Design review of the part built by this model. Coordinates are the model's own, in mm. A direction names the side the tool comes from. Round coordinates to 2 decimals unless told otherwise and drop trailing zeros. Order: outer loops, then holes, each group sorted by start corner. A loop starts at its lowest first (then second) coordinate and runs counter-clockwise, first axis right, second up. Notation, with made-up numbers: M 61,42.5 L 114,42.5 A14 ccw 114,51.5 Z; hole C -21.75,34 d8. An arc over 180 degrees is marked long. Write each question's results on one line, items separated by ' | '. Start each with the question number.
Item 1: Clearance check with flat-ended pins moving along their axes: pin 1 (1.5 mm diameter, centred on x = -3.5, y = 114, fed in from -Z); pin 2 (10 mm diameter, centred on x = 7, y = 132, fed in from +Z); pin 3 (5 mm diameter, centred on x = -8.5, y = 6.5, fed in from +Z); pin 4 (9 mm diameter, centred on x = -0.5, z = -3, fed in from -Y). State where each tip first meets the part, or that it passes through.
Item 2: Machinability: for faces 1 (the flat face through (10, -10, 0)), 2 (the flat face through (1, 0, -11)), 3 (the cylindrical face through (-1.951, -28.786, 19.86)), 4 (the flat face through (0, -8, -10)), 5 (the cylindrical face through (0.66, 93.67, -14.985)), which of the approach directions +Z, -Z, +X, -X, +Y, -Y give a long, thin tool a straight path to every point of the face, cutting with its end or side? Answer none if there is none.
Item 3: Wall thickness on line 1 (X direction, y = -5.5, z = -6); line 2 (Y direction, x = 2, z = -11.5); line 3 (Z direction, x = 0.5, y = 38): over which ranges is each line inside the solid? List them lowest first. Write a range as [from, to].
Item 4: Take a section at B-B, the plane x = 0. Write out the cut boundary in (y, z), plus the area to 3 significant figures.
Item 5: Take a section at C-C, the plane y = 39. Write out the cut boundary in (x, z).
Item 6: Take a section at D-D, the plane z = -19. Write out the cut boundary in (x, y).
Item 7: Take a section at A-A, the plane z = 0. Write out the cut boundary in (x, y), plus the area to 3 significant figures.
```python
from build123d import *

# Parameters (mm, degrees)
SKETCH_1_R           = 15
EXTRUDE_1_DEPTH      = 190
EXTRUDE_2_DEPTH      = 10
EXTRUDE_2_DEPTH_BACK = 10
EXTRUDE_3_DEPTH      = 20
EXTRUDE_3_DEPTH_BACK = 40
SKETCH_3_R           = 9


with BuildPart() as part:
    # 草图1 → 凸台-拉伸1 (new body)
    with BuildSketch(Plane(origin=(0, 0, 0), x_dir=(1, 0, 0), z_dir=(0, 1, 0))):
        with Locations(Location((0, 0, 0), (0, 0, 270))):
            Circle(SKETCH_1_R)
    extrude(amount=EXTRUDE_1_DEPTH)

    # 草图2 → 凸台-拉伸2 (add, two sides: drawn at the far end of the back side and taken through both)
    with BuildSketch(Plane.XY.offset(-EXTRUDE_2_DEPTH_BACK)):
        with BuildLine():
            Line((10, 0), (10, -20))
            ThreePointArc((10, -20), (0, -30), (-10, -20))
            Line((-10, -20), (-10, 0))
            ThreePointArc((-10, 0), (0, 10), (10, 0))
        make_face()
    extrude(amount=EXTRUDE_2_DEPTH + EXTRUDE_2_DEPTH_BACK)

    # 草图3 → 凸台-拉伸3 (add, two sides: drawn at the far end of the back side and taken through both)
    with BuildSketch(Plane.XY.offset(10).offset(-EXTRUDE_3_DEPTH_BACK)):
        with Locations((0, -20)):
            Circle(SKETCH_3_R)
    extrude(amount=EXTRUDE_3_DEPTH + EXTRUDE_3_DEPTH_BACK)


solid = part.part
```
Results list:
1) pin 1: z = -14.75 | pin 2: z = 14.87 | pin 3: z = 13.75 | pin 4: y = -30
2) face 1: +Z, -Z, +X, -Y | face 2: none | face 3: +Z | face 4: -Z | face 5: +Y
3) line 1: [-10, 10] | line 2: [-28.77, -11.23], [0, 190] | line 3: [-14.99, 14.99]
4) outline: M -30,-10 L -29,-10 L -29,-30 L -11,-30 L -11,-10 L 0,-10 L 0,-15 L 190,-15 L 190,15 L 0,15 L 0,10 L -11,10 L -11,30 L -29,30 L -29,10 L -30,10 Z | area: 7,020 mm²
5) outline: C 0,0 d30
6) outline: C 0,-20 d18
7) outline: M -15,0 L -10,0 L -10,-20 A10 ccw 10,-20 L 10,0 L 15,0 L 15,190 L -15,190 Z | area: 6,260 mm²
